Read the model definition and answer for the solid it produces. Units are mm, in the model's axes. A direction names the side the tool comes from. Give positions to 0.01 mm unless a question says otherwise; leave off trailing zeros. Write each loop counter-clockwise with the first axis right and the second up, starting at its lowest first coordinate (ties: lowest second). Pieces come first, ordered by that corner, then holes. Notation, with made-up numbers: (8, 50.5) - (31, 50.5) arc R17 cw to (31, 57.5) - close; hole circle Ø9 at (24.5, 46). An arc over 180 degrees is marked (long way). Answer as CSV lines item,"result".
```python
from build123d import *

# Parameters (mm, degrees)
BASE_PLATE_14MM_WITH_U_SLOT_DEPTH = 7
RAISED_BLOCK_18MM_DEPTH           = 9
STEP_CUT_SKETCH_W                 = 9
STEP_CUT_SKETCH_H                 = 8
STEP_CUT_DEPTH                    = 73.855407245


with BuildPart() as part:
    # Base Plate Profile Sketch → Base Plate 14mm with U-Slot (new, symmetric)
    with BuildSketch(Plane(origin=(0, 0, 0), x_dir=(1, 0, 0), z_dir=(0, 1, 0))):
        with BuildLine():
            Line((0, 23), (0, -23))
            Line((0, -23), (26, -23))
            Line((26, -23), (62.280898876, -18))
            Line((62.280898876, -18), (62.280898876, -7))
            Line((62.280898876, -7), (40.280898876, -7))
            ThreePointArc((40.280898876, -7), (33.280898876, 0), (40.280898876, 7))
            Line((40.280898876, 7), (62.280898876, 7))
            Line((62.280898876, 7), (62.280898876, 18))
            Line((62.280898876, 18), (26, 23))
            Line((26, 23), (0, 23))
        make_face()
    extrude(amount=BASE_PLATE_14MM_WITH_U_SLOT_DEPTH, both=True)

    # Raised Block Sketch → Raised Block 18mm (add, symmetric)
    with BuildSketch(Plane.ZY):
        Polygon((-23, 7), (-23, 16), (-7, 23), (7, 23), (23, 16), (23, 7), (23, -7), (-23, -7), align=None)
    extrude(amount=RAISED_BLOCK_18MM_DEPTH, both=True)

    # Step Cut Sketch → Step Cut (cut, through all)
    with BuildSketch(Plane(origin=(0, 23, 0), x_dir=(1, 0, 0), z_dir=(0, 1, 0))):
        with Locations((-4.5, 19)):
            Rectangle(STEP_CUT_SKETCH_W, STEP_CUT_SKETCH_H)
        with Locations((-4.5, -19)):
            Rectangle(STEP_CUT_SKETCH_W, STEP_CUT_SKETCH_H)
    extrude(amount=-STEP_CUT_DEPTH, mode=Mode.SUBTRACT)


solid = part.part
```
(1) A cutting plane is placed at C-C (y = -0.75). Write down the section's boundary in (x, z).
Worked out:
outline,"(-9, -15) - (0, -15) - (0, -23) - (26, -23) - (62.28, -18) - (62.28, -7) - (40.28, -7) arc R7 cw to (40.28, 7) - (62.28, 7) - (62.28, 18) - (26, 23) - (0, 23) - (0, 15) - (-9, 15) - close"
(2) For faces 1 (the flat face through (43.886, 0.098, 20.535)), 2 (the flat face through (0, 6, -19)), 3 (the flat face through (44.394, 0.098, -20.465)), 4 (the flat face through (29, 7, 0)), 5 (the flat face through (-5, 6, 15)), determine the directions among +Z, -Z, +X, -X, +Y, -Y from which every point of the face is accessible in a straight line to the end or side of a thin tool.
Worked out:
face 1,"+Z, +X, +Y, -Y"
face 2,"-Z, -X, +Y, -Y"
face 3,"-Z, +X, +Y, -Y"
face 4,"+Z, -Z, +X, +Y"
face 5,"+Z, -X, +Y, -Y"
(3) A cutting plane is placed at A-A (x = 54). Write down the section's boundary in (y, z).
Worked out:
outline,"(-7, -19.14) - (7, -19.14) - (7, -7) - (-7, -7) - close; (-7, 7) - (7, 7) - (7, 19.14) - (-7, 19.14) - close"
(4) A cutting plane is placed at D-D (x = 1). Write down the section's boundary in (y, z).
Worked out:
outline,"(-7, -23) - (16, -23) - (23, -7) - (23, 7) - (16, 23) - (-7, 23) - close"
(5) A cutting plane is placed at B-B (z = 0). Write down the section's boundary in (x, y), and give its area (3 significant figures).
Worked out:
outline,"(-9, -7) - (33.28, -7) - (33.28, 7) - (9, 7) - (9, 23) - (-9, 23) - close"
area,"880 mm^2"
(6) The mould has two halves that part along Z. Classify faces 6 (the flat face through (9, 13, 0)), 7 (the flat face through (1.87, 20.23, -13.33)), 8 (the flat face through (51, 0, -7)): +Z half, -Z half, draft (parallel to the pull), parting line (faces both ways), or undercut.
Worked out:
face 6,"draft"
face 7,"-Z half"
face 8,"undercut"
(7) Each of these flat-tipped pins is pushed along its axis until it touches: P1, Ø17.5, axis at y = 18.5, z = -6.5, coming from the +X side; P2, Ø4, axis at x = 47, z = -15, coming from the +Y side; P3, Ø2.5, axis at y = 10.5, z = -17.5, coming from the -X side; P4, Ø3, axis at x = 10, z = -4.5, coming from the +Y side. Where does it stop, or does it pass through?
Worked out:
P1,"stops at x = 9"
P2,"stops at y = 7"
P3,"stops at x = 0"
P4,"stops at y = 23"
(8) Find the intervals of material crossed by L1, parallel to Z at x = -5, y = 14; L2, parallel to X at y = 2, z = -17; L3, parallel to Y at x = 33, z = -4, in increasing order.
Worked out:
L1,"z = -15 to 15"
L2,"x = 0 to 62.28"
L3,"y = -7 to 7"
